```python
from build123d import *

# Parameters (mm, degrees)
SKETCH1_W               = 30
SKETCH1_H               = 30
BOSS_EXTRUDE1_DEPTH     = 180
SKETCH5_W               = 25
SKETCH5_H               = 25
CUT_EXTRUDE4_DEPTH      = 182.245689604
CUT_EXTRUDE3_DEPTH      = 184.098334236
CUT_EXTRUDE3_DEPTH_BACK = 10


with BuildPart() as part:
    # Sketch1 → Boss-Extrude1 (new body)
    with BuildSketch(Plane.XY):
        Rectangle(SKETCH1_W, SKETCH1_H)
    extrude(amount=BOSS_EXTRUDE1_DEPTH)

    # Sketch5 → Cut-Extrude4 (cut, through all)
    with BuildSketch(Plane(origin=(0, 0, 0), x_dir=(-1, 0, 0), z_dir=(0, 0, -1))):
        Rectangle(SKETCH5_W, SKETCH5_H)
    extrude(amount=-CUT_EXTRUDE4_DEPTH, mode=Mode.SUBTRACT)

    # Sketch3 → Cut-Extrude3 (cut, two sides: drawn at the far end of the back side and taken through both)
    with BuildSketch(Plane.XZ.offset(15).offset(-CUT_EXTRUDE3_DEPTH_BACK)):
        Polygon((-389.965751818, 130), (-15, 130), (15, 130), (15, 180), (15, 554.965751818), (-527.902959777, 1072.318278062), (-932.868711595, 647.352526244), align=None)
    extrude(amount=CUT_EXTRUDE3_DEPTH + CUT_EXTRUDE3_DEPTH_BACK, mode=Mode.SUBTRACT)


solid = part.part
```
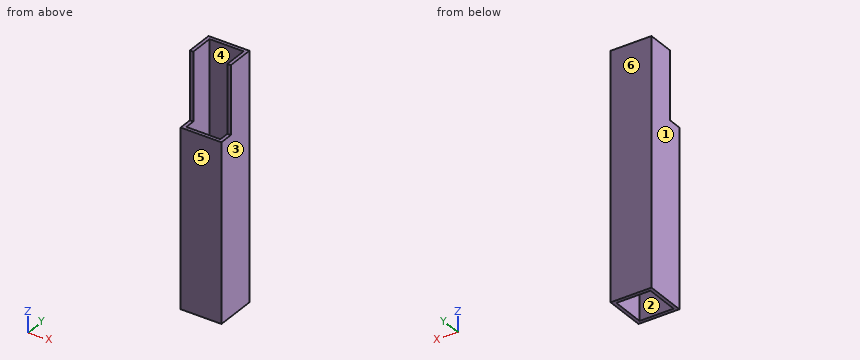
Verification items for the finished model (mm, model axes). Face numbers are marked on the shaded views. A direction names the side the tool comes from. Give positions to 0.01 mm unless a question says otherwise; leave off trailing zeros. Write each loop counter-clockwise with the first axis right and the second up, starting at its lowest first coordinate (ties: lowest second). Pieces come first, ordered by that corner, then holes. Notation, with made-up numbers: (-33, 34.5) - (22, 34.5) arc R24 cw to (22, 56.5) - close; hole circle Ø11 at (37.25, -31). An arc over 180 degrees is marked (long way). Put each result on its own line as item: value.
Q1. Set-up check for the marked faces 1 and 2: record each of +Z, -Z, +X, -X, +Y, -Y from which the full face is reachable in a straight line by a thin tool's end or side.
Result:
face 1: +Z, -Z, -X, +Y, -Y
face 2: +Z, -Z
Q2. Depth check by flat-ended pin: P1, Ø0.8, axis at x = -13.5, z = 148.5, coming from the -Y side; P2, Ø8, axis at x = -1, y = -12, coming from the +Z side. Enter the tip coordinate at first touch or a pass-through.
Result:
P1: y = -5
P2: z = 130
Q3. Section check B-B on x = -7.25. Record the cut outline in (y, z).
Result:
outline: (-15, 0) - (-12.5, 0) - (-12.5, 130) - (-15, 130) - close; (12.5, 0) - (15, 0) - (15, 180) - (12.5, 180) - close
Q4. Mould release check, pull along Y, two halves, no side actions. Record for the marked faces 3, 4, 5 and 6: released by +Y, released by -Y, zero draft, split by the parting line, or undercut.
Result:
face 3: zero draft
face 4: undercut
face 5: released by -Y
face 6: released by +Y
Q5. Section check A-A on y = -10.5. Record the cut outline in (x, z).
Result:
outline: (-15, 0) - (-12.5, 0) - (-12.5, 130) - (-15, 130) - close; (12.5, 0) - (15, 0) - (15, 130) - (12.5, 130) - close
Q6. Scan lines: probe 1 along X at (y, z) = (-1.5, 78); probe 2 along Z at (x, y) = (9.5, -13). Record each from-to range of solid material in increasing order. Write a range as from..to.
Result:
probe 1: -15..-12.5, 12.5..15
probe 2: 0..130
Q7. Section check D-D on z = 41.5. Record the cut outline in (x, y).
Result:
outline: (-15, -15) - (15, -15) - (15, 15) - (-15, 15) - close; hole (-12.5, -12.5) - (12.5, -12.5) - (12.5, 12.5) - (-12.5, 12.5) - close
Q8. Section check C-C on z = 131.5. Record the cut outline in (x, y).
Result:
outline: (-15, -5) - (-12.5, -5) - (-12.5, 12.5) - (12.5, 12.5) - (12.5, -5) - (15, -5) - (15, 15) - (-15, 15) - close
